For this review, use the dimensioned drawing (mm, ordinates from the lowest corner) and the shaded views. A direction names the side the tool comes from. Give positions to 0.01 mm unless a question says otherwise; leave off trailing zeros. Order: outer loops, then holes, each group sorted by start corner. A loop starts at its lowest first (then second) coordinate and runs counter-clockwise, first axis right, second up. Notation, with made-up numbers: M 63.25,37.5 L 116.25,37.5 A32 cw 116.25,75.5 Z; hole C -28.75,-27 d1. An arc over 180 degrees is marked long. Use CSV: the item, a comma, the result in double quotes. Start each with the question number.
(1) Consider section D-D (y = 13.5). Write out the cut boundary in (x, z), and give its area (3 significant figures).
(2) Consider section B-B (z = 10). Write out the cut boundary in (x, y), and give its area (3 significant figures).
(3) Clearance check with flat-ended pins moving along their axes: P1, Ø10, axis at y = 11, z = 11, coming from the -X side; P2, Ø5, axis at x = 6.5, z = 10, coming from the +Y side; P3, Ø7.5, axis at x = 67.5, z = 11.5, coming from the +Y side; P4, Ø1, axis at x = 29, z = 8.5, coming from the -Y side. State where each tip first meets the part, or that it passes through.
(4) Draft analysis for pull direction X (two halves, no side actions). For the marked faces 5, 6, 7 and 8, state which applies: pulls with the +X half, pulls with the -X half, needs draft (parallel to the pull), parting line crosses it, or undercut.
(5) Tool access review of the marked faces 1, 2, 3 and 4: name each direction out of +Z, -Z, +X, -X, +Y, -Y from which nothing blocks a thin tool from reaching the whole face with its end or side.
(6) Consider section C-C (x = 66.5). Write out the cut boundary in (y, z), and give its area (3 significant figures).
(7) Consider section A-A (y = 4.25). Write out the cut boundary in (x, z).
(8) Wall thickness on L1, parallel to X at y = 3.5, z = 10; L2, parallel to X at y = 2, z = 17.75; L3, parallel to Y at x = 9.5, z = 4: over which ranges is each line inside the solid? List them lowest first. Write a range as from..to.
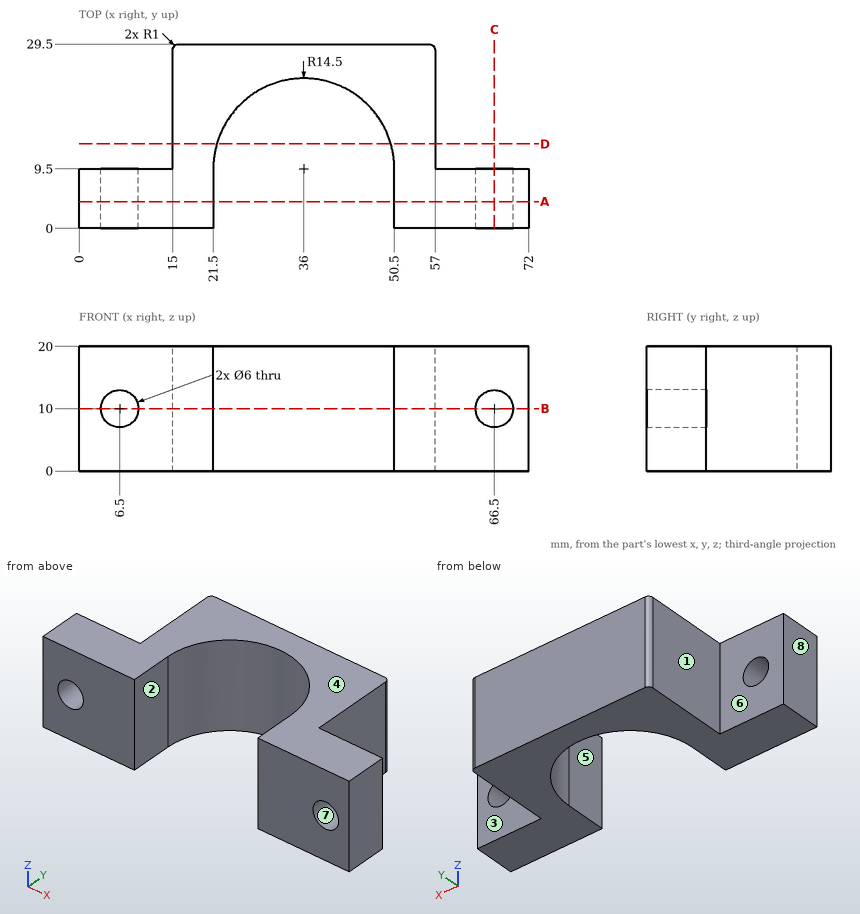
Check result:
1,outline,"M 15,0 L 22.06,0 L 22.06,20 L 15,20 Z; M 49.94,0 L 57,0 L 57,20 L 49.94,20 Z"
1,area,"283 mm^2"
2,outline,"M 0,0 L 3.5,0 L 3.5,9.5 L 0,9.5 Z; M 9.5,0 L 21.5,0 L 21.5,9.5 A14.5 cw 50.5,9.5 L 50.5,0 L 63.5,0 L 63.5,9.5 L 57,9.5 L 57,28.5 A1 ccw 56,29.5 L 16,29.5 A1 ccw 15,28.5 L 15,9.5 L 9.5,9.5 Z; M 69.5,0 L 72,0 L 72,9.5 L 69.5,9.5 Z"
2,area,"804 mm^2"
3,P1,"stops at x = 0"
3,P2,"passes through"
3,P3,"stops at y = 9.5"
3,P4,"stops at y = 21.91"
4,face 5,"undercut"
4,face 6,"needs draft"
4,face 7,"undercut"
4,face 8,"pulls with the -X half"
5,face 1,"+Z, -Z, -X, +Y"
5,face 2,"+Z, -Z, -Y"
5,face 3,"+Z, -Z, +X, +Y"
5,face 4,"+Z, +X, -X, +Y, -Y"
6,outline,"M 0,0 L 9.5,0 L 9.5,7 L 0,7 Z; M 0,13 L 9.5,13 L 9.5,20 L 0,20 Z"
6,area,"133 mm^2"
7,outline,"M 0,0 L 21.5,0 L 21.5,20 L 0,20 Z; M 50.5,0 L 72,0 L 72,20 L 50.5,20 Z; hole C 6.5,10 d6; hole C 66.5,10 d6"
8,L1,"x = 0..3.5, 9.5..21.5, 50.5..63.5, 69.5..72"
8,L2,"x = 0..21.5, 50.5..72"
8,L3,"y = 0..9.5"
